Design review of the part built by this model. Coordinates are the model's own, in mm. Give positions to 0.01 mm unless a question says otherwise; leave off trailing zeros. Loops run counter-clockwise (first coordinate to the right, second up) from the corner with the lowest first, then second, coordinate; pieces in that order, holes last. Notation, with made-up numbers: (74.5, -4.5) -> (122.5, -4.5) arc R12 cw to (122.5, 6.5) -> close; hole circle Ø3 at (76, -10.5). An arc over 180 degrees is marked (long way). Answer in a Markdown table with one row per item. Add a question column.
(1) Consider section A-A on x = 20. Write out the cut boundary in (y, z), then the cut area to 4 significant figures.
(2) Consider section B-B on y = 45. Write out the cut boundary in (x, z), then the cut area to 4 significant figures.
(3) For line 1 (Y direction, x = 20, z = 2.9); line 2 (X direction, y = 46.5, z = 0.3); line 3 (Y direction, x = 101.5, z = 2.1), list the stretches that pass through material, from the lowest coordinate up.
(4) For pin 1 (3.5 mm diameter, centred on x = 100, y = 45, fed in from -Z), flat-tipped, find the tip position at first contact; note if it passes through.
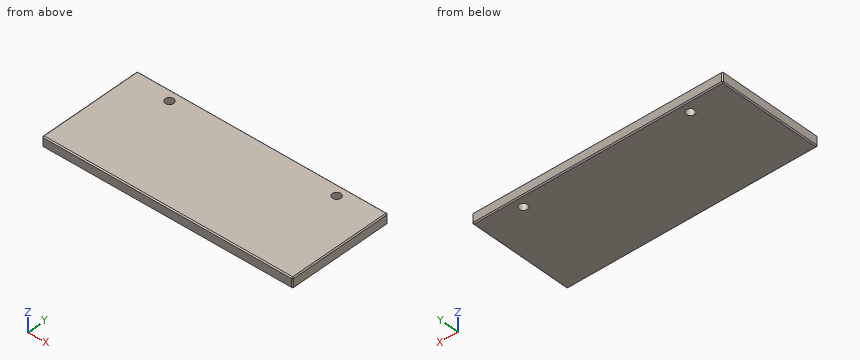
from build123d import *

# Parameters (mm, degrees)
SKETCH1_W                 = 120
SKETCH1_H                 = 50
BOSS_EXTRUDE1_DEPTH       = 5
F_4_0MM_DOWEL_HOLE1_D     = 4
F_4_0MM_DOWEL_HOLE1_DEPTH = 12
F_4_0MM_DOWEL_HOLE1_TIP   = 1.201721238
CHAMFER1_SIZE             = 0.5


with BuildPart() as part:
    # Sketch1 → Boss-Extrude1 (new body)
    with BuildSketch(Plane.XY):
        with Locations((60, 25)):
            Rectangle(SKETCH1_W, SKETCH1_H)
    extrude(amount=BOSS_EXTRUDE1_DEPTH)

    # Ø4.0mm dowel hole1
    with Locations(Plane.XY.offset(5)):
        with Locations((20, 45), (100, 45)):
            Hole(F_4_0MM_DOWEL_HOLE1_D / 2, depth=F_4_0MM_DOWEL_HOLE1_DEPTH)
            with Locations((0, 0, -(F_4_0MM_DOWEL_HOLE1_DEPTH + F_4_0MM_DOWEL_HOLE1_TIP / 2))):  # 118° drill point
                Cone(0, F_4_0MM_DOWEL_HOLE1_D / 2, F_4_0MM_DOWEL_HOLE1_TIP, mode=Mode.SUBTRACT)

    # Chamfer1
    chamfer1_edges = [part.edges().sort_by_distance(p)[0] for p in [
        (120, 25, 5),
        (60, 50, 5),
        (0, 25, 5),
        (60, 50, 0),
        (120, 25, 0),
        (60, 0, 0),
        (0, 25, 0),
        (0, 50, 2.5),
        (120, 50, 2.5),
        (120, 0, 2.5),
        (0, 0, 2.5),
        (60, 0, 5),
    ]]
    chamfer(chamfer1_edges, length=CHAMFER1_SIZE)


solid = part.part
Values follow:
| question | item | result |
|---|---|---|
| 1 | outline | (0, 0.5) -> (0.5, 0) -> (43, 0) -> (43, 5) -> (0.5, 5) -> (0, 4.5) -> close; (47, 0) -> (49.5, 0) -> (50, 0.5) -> (50, 4.5) -> (49.5, 5) -> (47, 5) -> close |
| 1 | area | 229.5 mm2 |
| 2 | outline | (0, 0.5) -> (0.5, 0) -> (18, 0) -> (18, 5) -> (0.5, 5) -> (0, 4.5) -> close; (22, 0) -> (98, 0) -> (98, 5) -> (22, 5) -> close; (102, 0) -> (119.5, 0) -> (120, 0.5) -> (120, 4.5) -> (119.5, 5) -> (102, 5) -> close |
| 2 | area | 559.5 mm2 |
| 3 | line 1 | 0 to 43, 47 to 50 |
| 3 | line 2 | 0.2 to 18.68, 21.32 to 98.68, 101.32 to 119.8 |
| 3 | line 3 | 0 to 43.68, 46.32 to 50 |
| 4 | pin 1 | through |
